Can you work these out from the drawing? Everything is in mm from the part's minimum corner. A direction names the side the tool comes from. Give positions to 0.01 mm unless a question says otherwise; leave off trailing zeros. Loops run counter-clockwise (first coordinate to the right, second up) from the corner with the lowest first, then second, coordinate; pieces in that order, holes last. Notation, with made-up numbers: (85.25, 77) - (91.25, 77) arc R9 ccw to (91.25, 87) - close; hole circle Ø11 at (33, -34). An arc over 180 degrees is marked (long way). Answer in a Markdown table with one row per item. Add a question column.
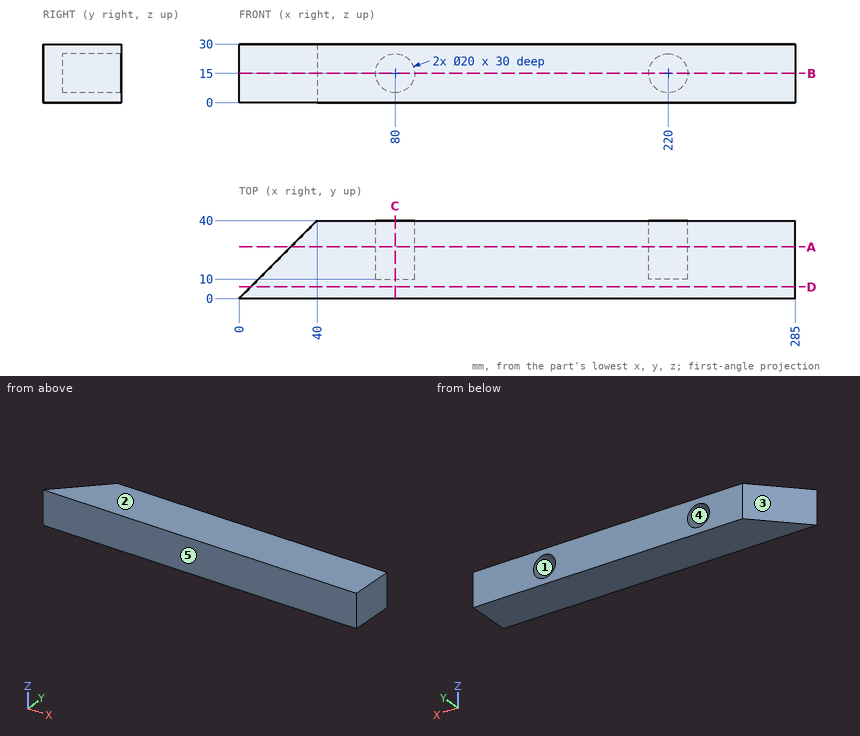
(1) On a 3-axis mill with a long thin cutter (end or side, diameter ignored), from which of +Z, -Z, +X, -X, +Y, -Y can I reach the whole of each face in a straight line? I mean the marked faces 1 and 2. Say none if no direction works.
(2) For pin 1 Ø4 at (x, z) = (82.5, 17) entering from +Y, with a flat end and sliding along its axis, tell me the tip position at first contact or that it passes through.
(3) Please list where these lines run through material, in increasing order: line 1 (Z direction, x = 80, y = 18); line 2 (X direction, y = 28, z = 15); line 3 (X direction, y = 26, z = 7).
(4) We'd pull the mould along X, two halves only. Please class the marked faces 3, 4 and 5: pulls with the +X half, pulls with the -X half, needs draft (parallel to the pull), parting line crosses it, or undercut.
(5) I want a section at D-D on y = 6. Please give me the cut outline in (x, z).
(6) I want a section at B-B on z = 15. Please give me the cut outline in (x, y), then the cut area to 3 significant figures.
(7) I want a section at C-C on x = 80. Please give me the cut outline in (y, z), then the cut area to 3 significant figures.
(8) I want a section at A-A on y = 26.5. Please give me the cut outline in (x, z).
Reported:
| question | item | result |
|---|---|---|
| 1 | face 1 | +Y |
| 1 | face 2 | +Z, +X, -X, +Y, -Y |
| 2 | pin 1 | y = 10 |
| 3 | line 1 | 0 to 5, 25 to 30 |
| 3 | line 2 | 28 to 70, 90 to 210, 230 to 285 |
| 3 | line 3 | 26 to 74, 86 to 214, 226 to 285 |
| 4 | face 3 | pulls with the -X half |
| 4 | face 4 | undercut |
| 4 | face 5 | needs draft |
| 5 | outline | (6, 0) - (285, 0) - (285, 30) - (6, 30) - close |
| 6 | outline | (0, 0) - (285, 0) - (285, 40) - (230, 40) - (230, 10) - (210, 10) - (210, 40) - (90, 40) - (90, 10) - (70, 10) - (70, 40) - (40, 40) - close |
| 6 | area | 9,400 mm² |
| 7 | outline | (0, 0) - (40, 0) - (40, 5) - (10, 5) - (10, 25) - (40, 25) - (40, 30) - (0, 30) - close |
| 7 | area | 600 mm² |
| 8 | outline | (26.5, 0) - (285, 0) - (285, 30) - (26.5, 30) - close; hole circle Ø20 at (80, 15); hole circle Ø20 at (220, 15) |
